Part model, mm, in its own coordinate system. Face numbers are marked on the shaded views. A direction names the side the tool comes from. Round coordinates to 2 decimals unless told otherwise and drop trailing zeros. Loops run counter-clockwise (first coordinate to the right, second up) from the corner with the lowest first, then second, coordinate; pieces in that order, holes last. Notation, with made-up numbers: M 14,60 L 39,60 A21 ccw 39,82 Z; hole C 55,31.5 d5. An arc over 180 degrees is marked long. Write each question's results on one line, items separated by ' | '.
from build123d import *

# Parameters (mm, degrees)
BOSS_EXTRUDE1_DEPTH = 75
SKETCH2_R           = 5.5
CUT_EXTRUDE1_DEPTH  = 45


with BuildPart() as part:
    # Sketch1 → Boss-Extrude1 (new body)
    with BuildSketch(Plane.XY):
        with BuildLine():
            Line((-15, 20), (15, 20))
            ThreePointArc((15, 20), (18.535533906, 18.535533906), (20, 15))
            Line((20, 15), (20, -15))
            ThreePointArc((20, -15), (18.535533906, -18.535533906), (15, -20))
            Line((15, -20), (-15, -20))
            ThreePointArc((-15, -20), (-18.535533906, -18.535533906), (-20, -15))
            Line((-20, -15), (-20, 15))
            ThreePointArc((-20, 15), (-18.535533906, 18.535533906), (-15, 20))
        make_face()
        with BuildLine():
            Line((-15, 16), (15, 16))
            ThreePointArc((15, 16), (15.707106781, 15.707106781), (16, 15))
            Line((16, 15), (16, -15))
            ThreePointArc((16, -15), (15.707106781, -15.707106781), (15, -16))
            Line((15, -16), (-15, -16))
            ThreePointArc((-15, -16), (-15.707106781, -15.707106781), (-16, -15))
            Line((-16, -15), (-16, 15))
            ThreePointArc((-16, 15), (-15.707106781, 15.707106781), (-15, 16))
        make_face(mode=Mode.SUBTRACT)
    extrude(amount=BOSS_EXTRUDE1_DEPTH)

    # Sketch2 → Cut-Extrude1 (cut)
    with BuildSketch(Plane(origin=(0, 0, 0), x_dir=(0, 0, 1), z_dir=(-0.7071067811865476, 0.7071067811865475, 0))):
        with Locations(Location((20, 0, 0), (0, 0, 319.997252237))):
            Circle(SKETCH2_R)
        with Locations(Location((55, 0, 0), (0, 0, 220.002747763))):
            Circle(SKETCH2_R)
    extrude(amount=-CUT_EXTRUDE1_DEPTH, mode=Mode.SUBTRACT)


solid = part.part
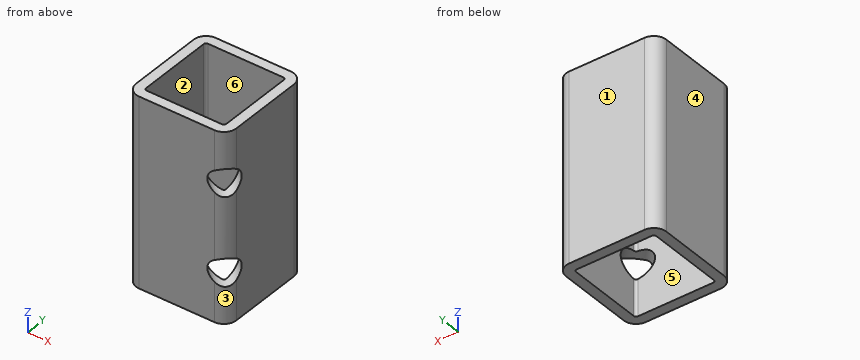
Item 1: Wall check: L1, parallel to X at y = 13, z = 28; L2, parallel to Z at x = 12.5, y = -18. Give the ranges that are in metal, low to high.
Filled sheet:
L1: -20 to -16, 16 to 20 | L2: 0 to 16.11, 23.89 to 51.11, 58.89 to 75
Item 2: Band-saw the part on A-A on y = 6.5. Give the cut face in (x, z), and give its area (3 significant figures).
Filled sheet:
outline: M -20,0 L -16,0 L -16,75 L -20,75 Z; M 16,0 L 20,0 L 20,75 L 16,75 Z | area: 600 mm^2
Item 3: Band-saw the part on C-C on z = 33.5. Give the cut face in (x, y).
Filled sheet:
outline: M -20,-15 A5 ccw -15,-20 L 15,-20 A5 ccw 20,-15 L 20,15 A5 ccw 15,20 L -15,20 A5 ccw -20,15 Z; hole M -16,-15 A1 ccw -15,-16 L 15,-16 A1 ccw 16,-15 L 16,15 A1 ccw 15,16 L -15,16 A1 ccw -16,15 Z
Item 4: Band-saw the part on D-D on z = 17. Give the cut face in (x, y).
Filled sheet:
outline: M -20,-15 A5 ccw -15,-20 L 13.48,-20 L 9.48,-16 L -15,-16 A1 cw -16,-15 L -16,15 A1 cw -15,16 L 15,16 A1 cw 16,15 L 16,-9.48 L 20,-13.48 L 20,15 A5 ccw 15,20 L -15,20 A5 ccw -20,15 Z
Item 5: Which spindle directions (+Z, -Z, +X, -X, +Y, -Y) get a long thin tool onto all of the face, cutting with end or side? Do the marked faces 1 and 2. Say none if no direction does.
Filled sheet:
face 1: +Z, -Z, +X, -X, +Y | face 2: +Z, -Z
Item 6: Two-plate mould, pull along Y, no slides. Class the marked faces 3, 4, 5 and 6: +Y half, -Y half, draft (parallel to the pull), parting line (faces both ways), or undercut.
Filled sheet:
face 3: -Y half | face 4: draft | face 5: undercut | face 6: undercut
